Could you check a few things on this model? Use its own coordinates, in mm. A direction names the side the tool comes from. Coordinates: 2 decimals unless noted, no trailing zeros. Loops run counter-clockwise (first coordinate to the right, second up) from the corner with the lowest first, then second, coordinate; pieces in that order, holes last. Notation, with made-up numbers: (13.5, 71) - (25.5, 71) arc R4 ccw to (25.5, 76) - close; hole circle Ø3 at (-15.5, 48). An arc over 180 degrees is marked (long way). Put each result on its own line as item: value. Start each with the question number.
```python
from build123d import *

# Parameters (mm, degrees)
EXTRUDE_1_DEPTH              = 15
HOLE_WIZARD_M4_1_D           = 3.3
HOLE_WIZARD_M4_1_DEPTH       = 9.5
HOLE_WIZARD_M4_1_TIP         = 0.991420021
HOLE_WIZARD_M6_1_D           = 5
HOLE_WIZARD_M6_1_DEPTH       = 12
HOLE_WIZARD_M6_1_CSINK_D     = 6.05
HOLE_WIZARD_M6_1_CSINK_ANGLE = 90
HOLE_WIZARD_M6_1_TIP         = 1.502151548


with BuildPart() as part:
    # 草图1 → 凸台-拉伸1 (new, symmetric)
    with BuildSketch(Plane.XY):
        with BuildLine():
            Line((-27.5, 58.5), (27.5, 58.5))
            Line((27.5, 58.5), (27.5, -17))
            Line((27.5, -17), (9, -17))
            Line((9, -17), (9, -13.228756555))
            ThreePointArc((9, -13.228756555), (0, 16), (-9, -13.228756555))
            Line((-9, -13.228756555), (-9, -17))
            Line((-9, -17), (-27.5, -17))
            Line((-27.5, -17), (-27.5, 58.5))
        make_face()
    extrude(amount=EXTRUDE_1_DEPTH, both=True)

    # M4 螺纹孔1
    with Locations(Plane.XY.offset(15)):
        with Locations((18.186533479, 10.5), (18.186533479, -10.5), (-18.186533479, -10.5), (-18.186533479, 10.5)):
            Hole(HOLE_WIZARD_M4_1_D / 2, depth=HOLE_WIZARD_M4_1_DEPTH)
            with Locations((0, 0, -(HOLE_WIZARD_M4_1_DEPTH + HOLE_WIZARD_M4_1_TIP / 2))):  # 118° drill point
                Cone(0, HOLE_WIZARD_M4_1_D / 2, HOLE_WIZARD_M4_1_TIP, mode=Mode.SUBTRACT)

    # M6 螺纹孔1
    with Locations(Plane(origin=(-20.5, 58.5, 8), x_dir=(0, 0, 1), z_dir=(0, 1, 0))):
        with Locations((0, 0), (-16, 0), (-16, 41), (0, 41)):
            CounterSinkHole(HOLE_WIZARD_M6_1_D / 2, HOLE_WIZARD_M6_1_CSINK_D / 2, depth=HOLE_WIZARD_M6_1_DEPTH, counter_sink_angle=HOLE_WIZARD_M6_1_CSINK_ANGLE)
            with Locations((0, 0, -(HOLE_WIZARD_M6_1_DEPTH + HOLE_WIZARD_M6_1_TIP / 2))):  # 118° drill point
                Cone(0, HOLE_WIZARD_M6_1_D / 2, HOLE_WIZARD_M6_1_TIP, mode=Mode.SUBTRACT)


solid = part.part
```
(1) I want a section at B-B on z = 0.75. List the corners of the cut face in (x, y) for me.
(2) I want a section at D-D on x = -12. List the corners of the cut face in (y, z) for me.
(3) I want a section at C-C on y = 54. List the corners of the cut face in (x, z) for me.
(4) Which directions (+Z, -Z, +X, -X, +Y, -Y) give clear straight access to the entire face, cutting with the end or side of a thin tool? Please do faces 5 (the cylindrical face through (22.61, 52.16, -9.34)), 6 (the flat face through (-18, -17, 0)), 7 (the cylindrical face through (-19.71, -11.13, 10.18)).
(5) For pin 1 Ø8 at (x, z) = (20.5, -8) entering from +Y; pin 2 Ø2.5 at (x, y) = (18.19, -10.5) entering from +Z, each with a flat end and sliding along its axis, tell me the tip position at first contact or that it passes through.
(6) I want a section at A-A on z = 12.5. List the corners of the cut face in (x, y) for me, and give its area (3 significant figures).
(7) I need wall thicknesses on L1, parallel to Z at x = -20.5, y = 53.25; L2, parallel to X at y = 52.5, z = -8; L3, parallel to X at y = 51, z = -8.75. Which ranges of each line are inside material? Lowest first, please. Write a range as [from, to].
(8) If we mould it in two halves opening along X, with no side actions, what happens to faces 1 (the conical face through (-17.92, -10.61, 4.68)), 2 (the flat face through (27.5, 21, 0)), 3 (the flat face through (0, 30, -15)), 4 (the flat face through (-27.5, 20, 0))? For each: pulls with the +X half, pulls with the -X half, needs draft (parallel to the pull), parting line crosses it, or undercut.
Answer sheet:
1. outline: (-27.5, -17) - (-9, -17) - (-9, -13.23) arc R16 cw (long way) to (9, -13.23) - (9, -17) - (27.5, -17) - (27.5, 58.5) - (-27.5, 58.5) - close
2. outline: (-17, -15) - (-10.58, -15) - (-10.58, 15) - (-17, 15) - close; (10.58, -15) - (58.5, -15) - (58.5, 15) - (10.58, 15) - close
3. outline: (-27.5, -15) - (27.5, -15) - (27.5, 15) - (-27.5, 15) - close; hole circle Ø5 at (-20.5, -8); hole circle Ø5 at (-20.5, 8); hole circle Ø5 at (20.5, -8); hole circle Ø5 at (20.5, 8)
4. face 5: +Y
4. face 6: +Z, -Z, +X, -X, -Y
4. face 7: +Z
5. pin 1: stops at y = 58.5
5. pin 2: stops at z = 5.26
6. outline: (-27.5, -17) - (-9, -17) - (-9, -13.23) arc R16 cw (long way) to (9, -13.23) - (9, -17) - (27.5, -17) - (27.5, 58.5) - (-27.5, 58.5) - close; hole circle Ø3.3 at (-18.19, -10.5); hole circle Ø3.3 at (-18.19, 10.5); hole circle Ø3.3 at (18.19, -10.5); hole circle Ø3.3 at (18.19, 10.5)
6. area: 3,280 mm^2
7. L1: z = [-15, -10.5], [-5.5, 5.5], [10.5, 15]
7. L2: x = [-27.5, -23], [-18, 18], [23, 27.5]
7. L3: x = [-27.5, -22.88], [-18.12, 18.12], [22.88, 27.5]
8. face 1: undercut
8. face 2: pulls with the +X half
8. face 3: needs draft
8. face 4: pulls with the -X half
